Here's how the part is built. I have some questions about the finished solid (model axes, mm). Face numbers are marked on the shaded views. A direction names the side the tool comes from. Coordinates: 2 decimals unless noted, no trailing zeros. Order: outer loops, then holes, each group sorted by start corner. A loop starts at its lowest first (then second) coordinate and runs counter-clockwise, first axis right, second up. Notation, with made-up numbers: (78, 49) -> (133, 49) arc R37 cw to (133, 86) -> close; hole circle Ø11 at (30, 12). An arc over 180 degrees is marked (long way). One line per item, written item: value. Start each with the question number.
```python
from build123d import *

# Parameters (mm, degrees)
SKETCH1_R           = 87.5
BOSS_EXTRUDE1_DEPTH = 700
SKETCH2_R           = 100
BOSS_EXTRUDE2_DEPTH = 600


with BuildPart() as part:
    # Sketch1 → Boss-Extrude1 (new, symmetric)
    with BuildSketch(Plane.XY):
        Circle(SKETCH1_R)
    extrude(amount=BOSS_EXTRUDE1_DEPTH, both=True)

    # Sketch2 → Boss-Extrude2 (add, symmetric)
    with BuildSketch(Plane.XY):
        Circle(SKETCH2_R)
    extrude(amount=BOSS_EXTRUDE2_DEPTH, both=True)


solid = part.part
```
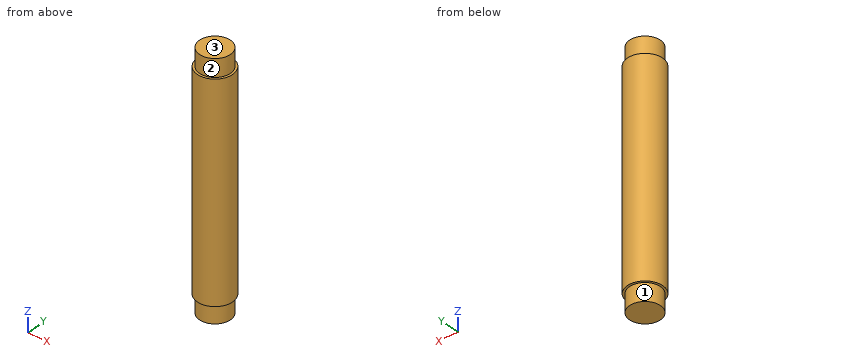
Q1. Imagine slicing it at C-C (z = -430). Write out the boundary of the cut face in (x, y), plus the area to 3 significant figures.
Q2. For P1, Ø1, axis at y = -37, z = 402.5, coming from the -X side; P2, Ø2, axis at y = 28.5, z = -235.5, coming from the +X side; P3, Ø6, axis at x = -64, y = -76.5, coming from the -Z side, each with a flat end and sliding along its axis, tell me the tip position at first contact or that it passes through.
Q3. Imagine slicing it at A-A (y = 0). Write out the boundary of the cut face in (x, z), plus the area to 3 significant figures.
Q4. For the marked faces 1, 2 and 3, which set-ups out of +Z, -Z, +X, -X, +Y, -Y let a thin tool reach every point of the face, with its end or its side?
Q5. I need wall thicknesses on line 1 (X direction, y = -0.5, z = -47.5); line 2 (X direction, y = 7, z = 454); line 3 (Y direction, x = -48, z = -428). Which ranges of each line are inside material? Lowest first, please.
Q6. Imagine slicing it at B-B (x = -51.5). Write out the boundary of the cut face in (y, z).
Completed:
1. outline: circle Ø200 at (0, 0)
1. area: 31,400 mm2
2. P1: stops at x = -93.1
2. P2: stops at x = 96.14
2. P3: stops at z = -600
3. outline: (-100, -600) -> (-87.5, -600) -> (-87.5, -700) -> (87.5, -700) -> (87.5, -600) -> (100, -600) -> (100, 600) -> (87.5, 600) -> (87.5, 700) -> (-87.5, 700) -> (-87.5, 600) -> (-100, 600) -> close
3. area: 275,000 mm2
4. face 1: -Z
4. face 2: +Z
4. face 3: +Z, +X, -X, +Y, -Y
5. line 1: x = -100 to 100
5. line 2: x = -99.75 to 99.75
5. line 3: y = -87.73 to 87.73
6. outline: (-85.72, -600) -> (-70.74, -600) -> (-70.74, -700) -> (70.74, -700) -> (70.74, -600) -> (85.72, -600) -> (85.72, 600) -> (70.74, 600) -> (70.74, 700) -> (-70.74, 700) -> (-70.74, 600) -> (-85.72, 600) -> close
